```python
from build123d import *

# Parameters (mm, degrees)
SKETCH2_R          = 12
SKETCH2_W          = 10
SKETCH2_H          = 14
CUT_EXTRUDE1_DEPTH = 5


with BuildPart() as part:
    # Sketch1 → Revolve1 (revolve)
    with BuildSketch(Plane.XY, mode=Mode.PRIVATE) as revolve1_sk:
        Polygon((-22.5, 0), (-22.5, 4.233), (-21.733, 5), (-5, 5), (-3.267949192, 6), (26.25, 6), (26.25, 12.5), (31.25, 12.5), (31.25, 0), align=None)
    revolve(revolve1_sk.sketch.rotate(Axis((31.25, 0, 0), (-1, 0, 0)), 270), axis=Axis((31.25, 0, 0), (-1, 0, 0)))

    # Sketch2 → Cut-Extrude1 (cut)
    with BuildSketch(Plane(origin=(0, 0, 0), x_dir=(0, 0, -1), z_dir=(1, 0, 0))):
        Circle(SKETCH2_R)
        Rectangle(SKETCH2_W, SKETCH2_H, mode=Mode.SUBTRACT)
    extrude(amount=-CUT_EXTRUDE1_DEPTH, mode=Mode.SUBTRACT)


solid = part.part
```
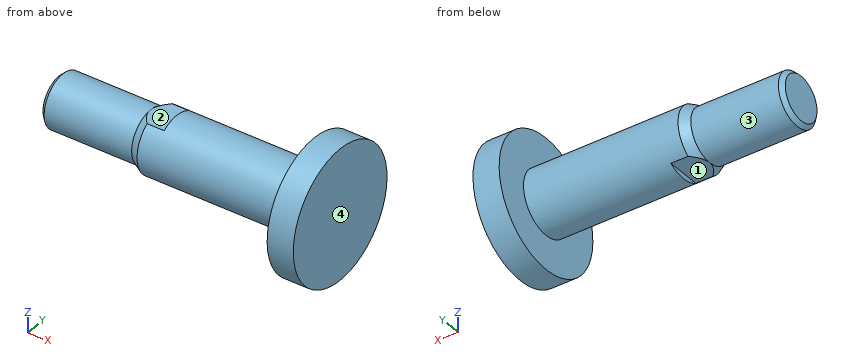
Build history of the part. All positions in model axes, mm. Face numbers are marked on the shaded views. A direction names the side the tool comes from. Coordinates: 2 decimals unless noted, no trailing zeros. Write each loop counter-clockwise with the first axis right and the second up, starting at its lowest first coordinate (ties: lowest second). Pieces come first, ordered by that corner, then holes.
1. Band-saw the part on C-C, the plane y = -7.75. Give the cut face in (x, z), and give its area (3 significant figures).
Answer block:
outline: (26.25, -9.81) - (31.25, -9.81) - (31.25, 9.81) - (26.25, 9.81) - close
area: 98.1 mm2
2. Drop flat-ended pins along their axis: pin 1 (4 mm diameter, centred on x = -2.5, y = -1, fed in from +Z); pin 2 (10 mm diameter, centred on x = 17, y = 7.5, fed in from -Z); pin 3 (0.5 mm diameter, centred on y = 1, z = 5.5, fed in from -X). Give the stop position or say it passes through.
Answer block:
pin 1: stops at z = 5
pin 2: stops at z = -5.45
pin 3: stops at x = 0
3. Band-saw the part on D-D, the plane z = -7.25. Give the cut face in (x, y), and give its area (3 significant figures).
Answer block:
outline: (26.25, -10.18) - (31.25, -10.18) - (31.25, 10.18) - (26.25, 10.18) - close
area: 102 mm2
4. Band-saw the part on A-A, the plane z = 0. Give the cut face in (x, y).
Answer block:
outline: (-22.5, -4.23) - (-21.73, -5) - (-5, -5) - (-3.27, -6) - (26.25, -6) - (26.25, -12.5) - (31.25, -12.5) - (31.25, 12.5) - (26.25, 12.5) - (26.25, 6) - (-3.27, 6) - (-5, 5) - (-21.73, 5) - (-22.5, 4.23) - close
5. 3-axis set-ups, long thin cutter, end or side, ignore diameter. For the marked faces 1, 2, 3 and 4: which of +Z, -Z, +X, -X, +Y, -Y reach the whole face in a straight line?
Answer block:
face 1: -Z, -X, +Y, -Y
face 2: +Z, -X, +Y, -Y
face 3: -X
face 4: +Z, -Z, +X, +Y, -Y
6. Drill centre lines: probe 1 along Z at (x, y) = (23.5, 4.25); probe 2 along X at (y, z) = (11, 4); probe 3 along Z at (x, y) = (-1.5, 0). Where is each one in solid material? Low to high.
Answer block:
probe 1: z = -4.24 to 4.24
probe 2: x = 26.25 to 31.25
probe 3: z = -5 to 5
7. Band-saw the part on B-B, the plane x = 14. Give the cut face in (y, z), and give its area (3 significant figures).
Answer block:
outline: circle Ø12 at (0, 0)
area: 113 mm2
